The model under review builds one solid part; all positions refer to its coordinate system, in mm. A direction names the side the tool comes from. Round coordinates to 2 decimals unless told otherwise and drop trailing zeros. Loops run counter-clockwise (first coordinate to the right, second up) from the corner with the lowest first, then second, coordinate; pieces in that order, holes last. Notation, with made-up numbers: M 48.25,73 L 64.25,73 A24 cw 64.25,104 Z; hole C 41.25,-16.5 d2. An arc over 180 degrees is marked long. Return JSON: item names as keys, results as strings. Group by question number.
Q1. Consider section C-C (y = 20.5). State the section outline as (x, z) points, and give its area (3 significant figures).
Q2. To check wall thickness, follow line 1 along X through (y, z) = (0, 1.1); line 2 along Y through (x, z) = (0, 1.15); line 3 along Y through (x, z) = (0, 0.5). State the ranges of each line that lie inside material, in increasing order.
Q3. Clearance check with flat-ended pins moving along their axes: pin 1 Ø1.8 at (x, z) = (-1, 4) entering from +Y; pin 2 Ø3 at (y, z) = (-26.5, 4.5) entering from -X; pin 3 Ø2 at (y, z) = (-34, 2) entering from +X. State where each tip first meets the part, or that it passes through.
Q4. Draft analysis for pull direction Y (two halves, no side actions). For faces 1 (the face through (10.655, 39.533, 1.839)), 2 (the face through (32.1, 18.4, 0.7)), 3 (the face through (-3.85, -41, 3)), state which applies: pulls with the +Y half, pulls with the -Y half, needs draft (parallel to the pull), parting line crosses it, or undercut.
Q5. Consider section B-B (x = 0). State the section outline as (y, z) points (3 decimals).
Q6. Consider section A-A (y = 0). State the section outline as (x, z) points, and give its area (3 significant figures).
Q7. For faces 4 (the face through (-37.257, -17.065, 2.797)), 5 (the face through (14.278, 38.412, 2.797)), 6 (the face through (-3.85, -25.5, 2.3)), list the 3-axis set-ups (+Z, -Z, +X, -X, +Y, -Y) from which the entire face can be reached by the end or side of a thin tool; tool diameter is ignored.
from build123d import *

# Parameters (mm, degrees)
SKETCH3_OUTSIDE_W   = 117.478
SKETCH3_OUTSIDE_H   = 117.478
CUT_EXTRUDE2_DEPTH  = 5.230463
SKETCH4_W           = 7.7
SKETCH4_H           = 1.5
BOSS_EXTRUDE1_DEPTH = 6


with BuildPart() as part:
    # Sketch2 → Boss-Revolve (revolve)
    with BuildSketch(Plane(origin=(0, 0, 0), x_dir=(0, 0, -1), z_dir=(1, 0, 0))):
        Polygon((-3.730461265, 45), (0, 37), (0, 0), (-1.5, 0), (-1.5, 37), (-5.230461265, 45), align=None)
    revolve(axis=Axis((0, 0, 0), (0, 0, 1)))

    # Sketch3 outside → Cut-Extrude2 (cut)
    # profile 1 of 2: a face of its own
    with BuildSketch(Plane.XY):
        Rectangle(SKETCH3_OUTSIDE_W, SKETCH3_OUTSIDE_H)
        with BuildLine():
            Line((-3.85, -36.799150805), (-3.85, -44.835003067))
            Line((-3.85, -44.835003067), (3.85, -44.835003067))
            Line((3.85, -44.835003067), (3.85, -36.799150805))
            ThreePointArc((3.85, -36.799150805), (29.354073591, -22.524172873), (36.541703472, 5.805506641))
            Line((36.541703472, 5.805506641), (44.303740708, 7.88533825))
            Line((44.303740708, 7.88533825), (42.31083406, 15.322967112))
            Line((42.31083406, 15.322967112), (34.548796825, 13.243135503))
            ThreePointArc((34.548796825, 13.243135503), (32.04293994, 18.5), (28.743290184, 23.298567969))
            Line((28.743290184, 23.298567969), (34.425495811, 28.980773595))
            Line((34.425495811, 28.980773595), (28.980773595, 34.425495811))
            Line((28.980773595, 34.425495811), (23.298567969, 28.743290184))
            ThreePointArc((23.298567969, 28.743290184), (18.5, 32.04293994), (13.243135503, 34.548796825))
            Line((13.243135503, 34.548796825), (15.322967112, 42.31083406))
            Line((15.322967112, 42.31083406), (7.88533825, 44.303740708))
            Line((7.88533825, 44.303740708), (5.805506641, 36.541703472))
            ThreePointArc((5.805506641, 36.541703472), (-29.354073591, 22.524172873), (-33.793999435, -15.065377598))
            Line((-33.793999435, -15.065377598), (-40.753251635, -19.083303729))
            Line((-40.753251635, -19.083303729), (-36.903251635, -25.751699338))
            Line((-36.903251635, -25.751699338), (-29.943999435, -21.733773207))
            ThreePointArc((-29.943999435, -21.733773207), (-26.162950904, -26.162950904), (-21.733773207, -29.943999435))
            Line((-21.733773207, -29.943999435), (-25.751699338, -36.903251635))
            Line((-25.751699338, -36.903251635), (-19.083303729, -40.753251635))
            Line((-19.083303729, -40.753251635), (-15.065377598, -33.793999435))
            ThreePointArc((-15.065377598, -33.793999435), (-9.576304669, -35.739255573), (-3.85, -36.799150805))
        make_face(mode=Mode.SUBTRACT)
    # profile 2 of 2: a face of its own
    with BuildSketch(Plane.XY):
        with BuildLine():
            Line((3.85, -28.238758825), (3.85, -24.5))
            Line((3.85, -24.5), (-3.85, -24.5))
            Line((-3.85, -24.5), (-3.85, -28.238758825))
            ThreePointArc((-3.85, -28.238758825), (0, 28.5), (3.85, -28.238758825))
        make_face()
    extrude(amount=CUT_EXTRUDE2_DEPTH, mode=Mode.SUBTRACT)

    # Sketch4 → Boss-Extrude1 (add)
    with BuildSketch(Plane.XY):
        with Locations((0, -25.25)):
            Rectangle(SKETCH4_W, SKETCH4_H)
    extrude(amount=BOSS_EXTRUDE1_DEPTH)


solid = part.part
Values:
{
 "1": {"outline": "M -30.8,0 L -19.8,0 L -19.8,1.5 L -30.8,1.5 Z; M 19.8,0 L 30.8,0 L 30.8,1.5 L 19.8,1.5 Z", "area": "33.0 mm2"},
 "2": {"line 1": "x = -37 to -28.5, 28.5 to 37", "line 2": "y = -39.47 to -24.5, 28.5 to 37", "line 3": "y = -38.07 to -24.5, 28.5 to 37"},
 "3": {"pin 1": "stops at y = -24.5", "pin 2": "stops at x = -37.34", "pin 3": "stops at x = 16.47"},
 "4": {"face 1": "pulls with the +Y half", "face 2": "undercut", "face 3": "needs draft"},
 "5": {"outline": "M -44.835,3.654 L -37,0 L -24.5,0 L -24.5,6 L -26,6 L -26,1.5 L -37,1.5 L -44.835,5.154 Z; M 28.5,0 L 37,0 L 37,1.5 L 28.5,1.5 Z"},
 "6": {"outline": "M -37,0 L -28.5,0 L -28.5,1.5 L -37,1.5 Z; M 28.5,0 L 37,0 L 37,1.5 L 28.5,1.5 Z", "area": "25.5 mm2"},
 "7": {"face 4": "+Z, -Z, -X", "face 5": "+Z, -Z, +X", "face 6": "+Z, -Z"}
}
